The listing builds one solid part. Answer for the finished solid, in the listing's coordinates (mm). Give positions to 0.01 mm unless a question says otherwise; leave off trailing zeros. Loops run counter-clockwise (first coordinate to the right, second up) from the corner with the lowest first, then second, coordinate; pieces in that order, holes last. Notation, with made-up numbers: M 81.25,45 L 133.25,45 A26 cw 133.25,74 Z; hole C 87.5,1 d9. An arc over 180 degrees is marked long. Return JSON: item names as keys, results as strings.
from build123d import *

# Parameters (mm, degrees)
SKETCH1_W                                       = 99
SKETCH1_H                                       = 99
BOSS_EXTRUDE1_DEPTH                             = 5
FILLET1_R                                       = 5
CSK_FOR_M3_FLAT_HEAD_MACHINE_SCREW1_D           = 3.2
CSK_FOR_M3_FLAT_HEAD_MACHINE_SCREW1_DEPTH       = 8.5
CSK_FOR_M3_FLAT_HEAD_MACHINE_SCREW1_CSINK_D     = 6.3
CSK_FOR_M3_FLAT_HEAD_MACHINE_SCREW1_CSINK_ANGLE = 90
CSK_FOR_M3_FLAT_HEAD_MACHINE_SCREW1_TIP         = 0.96137699


with BuildPart() as part:
    # Sketch1 → Boss-Extrude1 (new body)
    with BuildSketch(Plane(origin=(0, 0, 0), x_dir=(1, 0, 0), z_dir=(0, 1, 0))):
        Rectangle(SKETCH1_W, SKETCH1_H)
    extrude(amount=BOSS_EXTRUDE1_DEPTH)

    # Fillet1
    fillet1_edges = [part.edges().sort_by_distance(p)[0] for p in [
        (49.5, 2.5, 49.5),
        (-49.5, 2.5, 49.5),
        (-49.5, 2.5, -49.5),
        (49.5, 2.5, -49.5),
    ]]
    fillet(fillet1_edges, radius=FILLET1_R)

    # CSK for M3 Flat Head Machine Screw1
    with Locations(Plane(origin=(0, 5, 0), x_dir=(1, 0, 0), z_dir=(0, 1, 0))):
        with Locations((-44.5, 44.5), (44.5, 44.5), (0, 46), (-46, 0), (-44.5, -44.5), (0, -46), (44.5, -44.5), (46, 0)):
            CounterSinkHole(CSK_FOR_M3_FLAT_HEAD_MACHINE_SCREW1_D / 2, CSK_FOR_M3_FLAT_HEAD_MACHINE_SCREW1_CSINK_D / 2, depth=CSK_FOR_M3_FLAT_HEAD_MACHINE_SCREW1_DEPTH, counter_sink_angle=CSK_FOR_M3_FLAT_HEAD_MACHINE_SCREW1_CSINK_ANGLE)
            with Locations((0, 0, -(CSK_FOR_M3_FLAT_HEAD_MACHINE_SCREW1_DEPTH + CSK_FOR_M3_FLAT_HEAD_MACHINE_SCREW1_TIP / 2))):  # 118° drill point
                Cone(0, CSK_FOR_M3_FLAT_HEAD_MACHINE_SCREW1_D / 2, CSK_FOR_M3_FLAT_HEAD_MACHINE_SCREW1_TIP, mode=Mode.SUBTRACT)


solid = part.part
(1) Given pin 1 (5 mm diameter, centred on x = -44.5, z = 44.5, fed in from +Y); pin 2 (4 mm diameter, centred on x = 0, z = 46, fed in from +Y), each flat-ended and moving along its own axis, determine where each tip first touches the part or whether it passes through.
Values follow:
{"pin 1": "y = 4.35", "pin 2": "y = 3.85"}
(2) Determine the mould class of faces 1 (the cylindrical face through (43.76, 1.7, 45.92)), 2 (the flat face through (-1, 5, -1)), 3 (the flat face through (-49.5, 2, 1)), 4 (the flat face through (49.5, 2, 1)) for opening direction X: released by +X, released by -X, zero draft, split by the parting line, or undercut.
Values follow:
{"face 1": "undercut", "face 2": "zero draft", "face 3": "released by -X", "face 4": "released by +X"}
(3) The part is cut by section B-B (z = 0). Determine the outline of the cut face in (x, y).
Values follow:
{"outline": "M -49.5,0 L -47.6,0 L -47.6,3.45 L -49.15,5 L -49.5,5 Z; M -44.4,0 L 44.4,0 L 44.4,3.45 L 42.85,5 L -42.85,5 L -44.4,3.45 Z; M 47.6,0 L 49.5,0 L 49.5,5 L 49.15,5 L 47.6,3.45 Z"}
(4) The part is cut by section A-A (x = 0). Determine the outline of the cut face in (y, z), and give its area (3 significant figures).
Values follow:
{"outline": "M 0,-49.5 L 5,-49.5 L 5,-49.15 L 3.45,-47.6 L 0,-47.6 Z; M 0,-44.4 L 3.45,-44.4 L 5,-42.85 L 5,42.85 L 3.45,44.4 L 0,44.4 Z; M 0,47.6 L 3.45,47.6 L 5,49.15 L 5,49.5 L 0,49.5 Z", "area": "458 mm²"}
(5) Straight lines are drawn through the part: line 1 along Z through (x, y) = (0, 0.8); line 2 along X through (y, z) = (2.05, -43.5); line 3 along Z through (x, y) = (45, 0.7). For each, find the intervals that lie inside material, in ascending order.
Values follow:
{"line 1": "-49.5 to -47.6, -44.4 to 44.4, 47.6 to 49.5", "line 2": "-49.5 to -45.75, -43.25 to 43.25, 45.75 to 49.5", "line 3": "-49.47 to -46.02, -42.98 to -1.25, 1.25 to 42.98, 46.02 to 49.47"}
